from build123d import *
from build123d.topology import SkipClean

# Parameters (mm, degrees)
SKETCH1_R           = 1.25
BOSS_EXTRUDE1_DEPTH = 1
SKETCH2_R           = 1
BOSS_EXTRUDE2_DEPTH = 1
BOSS_EXTRUDE3_DEPTH = 2
SKETCH4_R           = 1
BOSS_EXTRUDE4_DEPTH = 1
BOSS_EXTRUDE5_START = 1
SKETCH5_R           = 1.25
BOSS_EXTRUDE5_DEPTH = 1
SKETCH6_R           = 1
BOSS_EXTRUDE6_DEPTH = 3


with BuildPart() as part:
    # Sketch1 → Boss-Extrude1 (new body)
    with BuildSketch(Plane.XY):
        Circle(SKETCH1_R)
    extrude(amount=-BOSS_EXTRUDE1_DEPTH)

    # Sketch2 → Boss-Extrude2 (add)
    with BuildSketch(Plane.XY):
        Circle(SKETCH2_R)
    extrude(amount=BOSS_EXTRUDE2_DEPTH)

    # Sketch3 → Boss-Extrude3 (add)
    with BuildSketch(Plane.XY.offset(1)):
        with BuildLine():
            Line((0, 0.5), (15, 0.995012469))
            ThreePointArc((15, 0.995012469), (16.099750623, 0), (15, -0.995012469))
            Line((15, -0.995012469), (0, -0.5))
            ThreePointArc((0, -0.5), (-0.5, 0), (0, 0.5))
        make_face()
    extrude(amount=BOSS_EXTRUDE3_DEPTH)

    # Sketch4 → Boss-Extrude4 (add)
    with SkipClean():  # the faces are left unmerged after this step: merging them gives an invalid solid
        with BuildSketch(Plane.XY.offset(3)):
            with Locations(Location((15.099750623, 0, 0), (0, 0, 264.275189548))):
                Circle(SKETCH4_R)
        extrude(amount=BOSS_EXTRUDE4_DEPTH)

    # Sketch5 → Boss-Extrude5 (add)
    with SkipClean():  # the faces are left unmerged after this step: merging them gives an invalid solid
        with BuildSketch(Plane.XY.offset(BOSS_EXTRUDE5_START)):
            Circle(SKETCH5_R)
        extrude(amount=-BOSS_EXTRUDE5_DEPTH)

    # Sketch6 → Boss-Extrude6 (add)
    with SkipClean():  # the faces are left unmerged after this step: merging them gives an invalid solid
        with BuildSketch(Plane(origin=(0, 0, -1), x_dir=(-1, 0, 0), z_dir=(0, 0, -1))):
            Circle(SKETCH6_R)
        extrude(amount=BOSS_EXTRUDE6_DEPTH)


solid = part.part
Geometry: final body of the model. Coordinates: model frame, mm. A direction names the side the tool comes from. Coordinates: 2 decimals unless noted, no trailing zeros. Order: outer loops, then holes, each group sorted by start corner. A loop starts at its lowest first (then second) coordinate and runs counter-clockwise, first axis right, second up.
(1) Section query D-D (x = 15.25). Return the cut outline in (y, z), plus the area to 3 significant figures.
(2) Material intervals for probe 1 along Z at (x, y) = (12, 0.7); probe 2 along Y at (x, z) = (15, 3); probe 3 along Z at (x, y) = (14.75, -0.1), sorted ascending.
(3) First-contact query: pin 1 (1 mm diameter, centred on x = 3, y = 0.5, fed in from +Z); pin 2 (1 mm diameter, centred on x = 10.5, y = 0, fed in from -Z); pin 3 (2 mm diameter, centred on x = 10, z = 1, fed in from +Y). Flat tips, straight axial feed; report the tip coordinate or a pass-through.
(4) Section query B-B (y = 0.7). Return the cut outline in (x, z).
(5) Section query A-A (y = 0). Return the cut outline in (x, z).
(6) Access query for faces 1 (the face through (-0.5, 0, 2)), 2 (the face through (0, -1, -2)), 3 (the face through (10, 0, 1)), 4 (the face through (15, 0, 4)). Directions: +Z, -Z, +X, -X, +Y, -Y. A direction counts if a zero-diameter tool reaches every point of the face in a straight line with its end or side. Return the directions, or none.
(7) Section query C-C (z = 2.25). Return the cut outline in (x, y), plus the area to 3 significant figures.
Solution:
1. outline: (-0.99, 1) - (0.99, 1) - (0.99, 4) - (-0.99, 4) - close
1. area: 5.93 mm2
2. probe 1: z = 1 to 3
2. probe 2: y = -1 to 1
2. probe 3: z = 1 to 4
3. pin 1: stops at z = 3
3. pin 2: stops at z = 1
3. pin 3: stops at y = 0.86
4. outline: (-1.04, -1) - (-0.71, -1) - (-0.71, -4) - (0.71, -4) - (0.71, -1) - (1.04, -1) - (1.04, 1) - (-1.04, 1) - close; (6.06, 1) - (15.81, 1) - (15.81, 4) - (14.39, 4) - (14.39, 3) - (6.06, 3) - close
5. outline: (-1.25, -1) - (-1, -1) - (-1, -4) - (1, -4) - (1, -1) - (1.25, -1) - (1.25, 1) - (16.1, 1) - (16.1, 4) - (14.1, 4) - (14.1, 3) - (-0.5, 3) - (-0.5, 1) - (-1.25, 1) - close
6. face 1: +Z, -X
6. face 2: -Z
6. face 3: -Z, +X, +Y, -Y
6. face 4: +Z, +X, -X, +Y, -Y
7. outline: (0, -0.5) - (15, -1) arc R1 ccw (long way) to (15, 1) - (0, 0.5) arc R0.5 ccw to start
7. area: 24.6 mm2
